Here's the drawing with two shaded views (mm, measured from the low corner). I have some questions. A direction names the side the tool comes from. Coordinates: 2 decimals unless noted, no trailing zeros. Write each loop counter-clockwise with the first axis right and the second up, starting at its lowest first coordinate (ties: lowest second). Pieces come first, ordered by that corner, then holes.
Item 1: I want a section at C-C on y = 57. Please give me the cut outline in (x, z).
Item 2: If I drill on probe 1 along Y at (x, z) = (250, 45); probe 2 along Z at (x, y) = (417, 332); probe 3 along X at (y, z) = (307, 46.5) (1 decimal), over which ranges is the centre line in solid material (lowest first)?
Item 3: Which directions (+Z, -Z, +X, -X, +Y, -Y) give clear straight access to the entire face, cutting with the end or side of a thin tool? Please do the marked faces 1 and 2.
Item 4: For P1, Ø12, axis at y = 440, z = 13.5, coming from the -X side, with a flat end and sliding along its axis, tell me the tip position at first contact or that it passes through.
Item 5: I want a section at A-A on x = 250. Please give me the cut outline in (y, z), then the cut area to 3 significant figures.
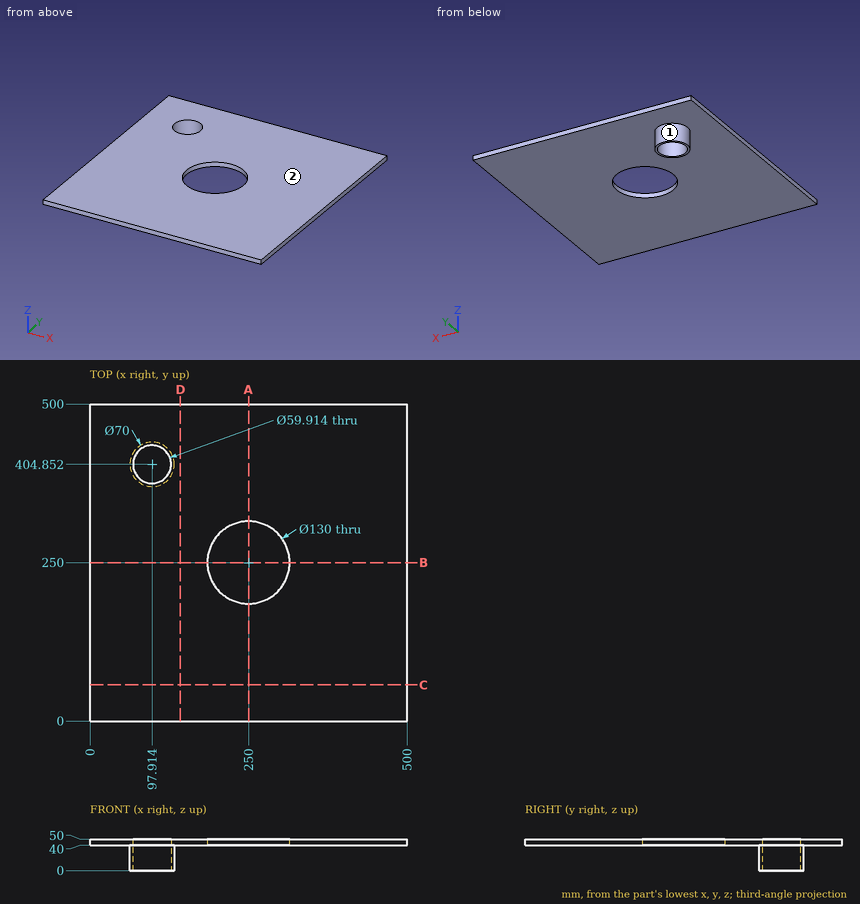
Response values:
1. outline: (0, 40) - (500, 40) - (500, 50) - (0, 50) - close
2. probe 1: y = 0 to 185, 315 to 500
2. probe 2: z = 40 to 50
2. probe 3: x = 0 to 218.8, 281.2 to 500
3. face 1: -Z
3. face 2: +Z, +X, -X, +Y, -Y
4. P1: stops at x = 78.54
5. outline: (0, 40) - (185, 40) - (185, 50) - (0, 50) - close; (315, 40) - (500, 40) - (500, 50) - (315, 50) - close
5. area: 3,700 mm2
